```python
from build123d import *

# Parameters (mm, degrees)
SKETCH1_R           = 85
SKETCH1_R_2         = 40
BOSS_EXTRUDE1_DEPTH = 10
CHAMFER1_SIZE       = 2


with BuildPart() as part:
    # Sketch1 → Boss-Extrude1 (new body)
    with BuildSketch(Plane(origin=(0, 0, 0), x_dir=(0, 0, -1), z_dir=(1, 0, 0))):
        Circle(SKETCH1_R)
        Circle(SKETCH1_R_2, mode=Mode.SUBTRACT)
    extrude(amount=BOSS_EXTRUDE1_DEPTH)

    # Chamfer1
    chamfer1_edges = [part.edges().sort_by_distance(p)[0] for p in [
        (0, 0, 85),
        (10, 0, 85),
        (10, 0, 40),
    ]]
    chamfer(chamfer1_edges, length=CHAMFER1_SIZE)


solid = part.part
```
CAD build for the part. Positions are in the model's coordinates, mm. Give positions to 0.01 mm unless a question says otherwise; leave off trailing zeros. Loops run counter-clockwise (first coordinate to the right, second up) from the corner with the lowest first, then second, coordinate; pieces in that order, holes last. Notation, with made-up numbers: (-8, 54) -> (51, 54) arc R21 cw to (51, 73) -> close; hole circle Ø2 at (-35.5, 34.5). An arc over 180 degrees is marked (long way). Use a Markdown table: item, result.
1. Flat gauge pins, fed straight in: pin 1 (6 mm diameter, centred on x = 6, y = 57.5, fed in from -Z); pin 2 (5 mm diameter, centred on x = 6, z = 53, fed in from -Y); pin 3 (5 mm diameter, centred on x = 2.5, z = -33, fed in from +Y). Where does each tip first touch, or does it go through?
Check result:
| item | result |
|---|---|
| pin 1 | stops at z = -65.23 |
| pin 2 | stops at y = -68.37 |
| pin 3 | stops at y = 79.34 |
2. Slice it at A-A (y = 0). List the corners of the cut face in (x, z).
Check result:
| item | result |
|---|---|
| outline | (0, -83) -> (2, -85) -> (8, -85) -> (10, -83) -> (10, -42) -> (8, -40) -> (0, -40) -> close; (0, 40) -> (8, 40) -> (10, 42) -> (10, 83) -> (8, 85) -> (2, 85) -> (0, 83) -> close |
3. Slice it at C-C (x = 4.25). List the corners of the cut face in (y, z).
Check result:
| item | result |
|---|---|
| outline | circle Ø170 at (0, 0); hole circle Ø80 at (0, 0) |
4. Mould opens along Z. For faces 1 (the flat face through (0, -36, 20)), 2 (the cylindrical face through (4.958, -51.721, 67.453)), 3 (the cylindrical face through (3.94, -39.05, 8.67)) say: pulls with the +Z half, pulls with the -Z half, needs draft (parallel to the pull), parting line crosses it, or undercut.
Check result:
| item | result |
|---|---|
| face 1 | needs draft |
| face 2 | parting line crosses it |
| face 3 | undercut |
5. Wall check: L1, parallel to Y at x = 4.75, z = 0; L2, parallel to Y at x = 9.5, z = -18.5; L3, parallel to Z at x = 5, y = 7. Give the ranges that are in metal, low to high. Write a range as [from, to].
Check result:
| item | result |
|---|---|
| L1 | y = [-85, -40], [40, 85] |
| L2 | y = [-81.42, -37.15], [37.15, 81.42] |
| L3 | z = [-84.71, -39.38], [39.38, 84.71] |
